Design review of the part shown in the three views and the two pictorial views. Dimensions are in mm from the part's minimum x, y and z. Round coordinates to 2 decimals unless told otherwise and drop trailing zeros. Order: outer loops, then holes, each group sorted by start corner. A loop starts at its lowest first (then second) coordinate and runs counter-clockwise, first axis right, second up.
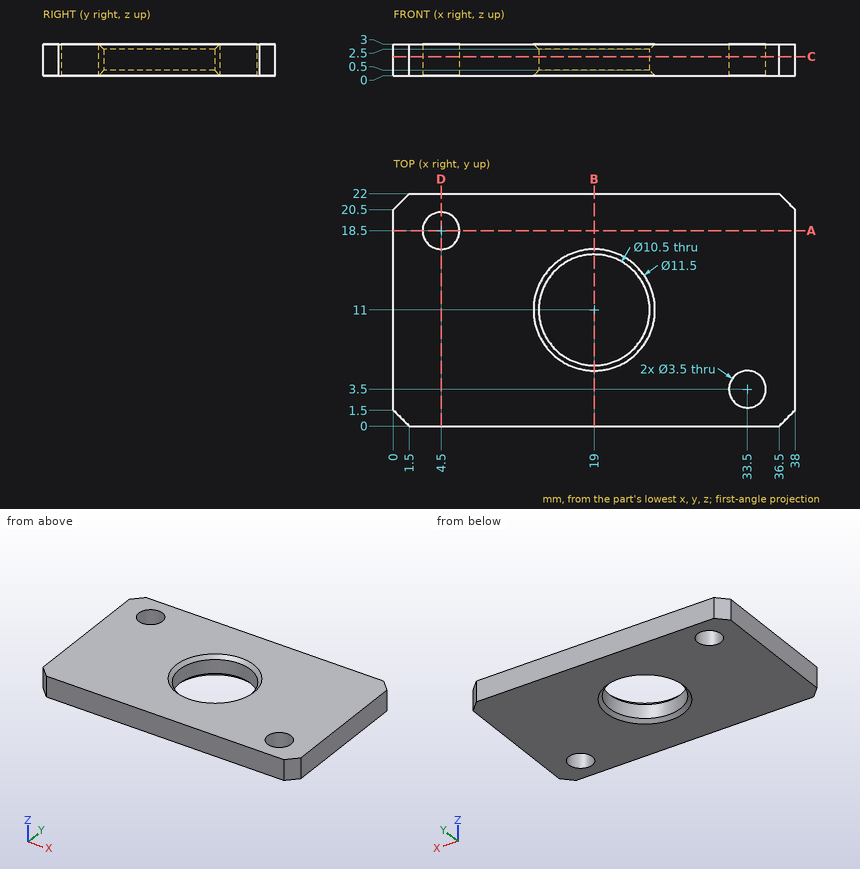
(1) Clearance check with a flat-ended pin moving along its axis: P1, Ø1, axis at x = 6, z = 0.5, coming from the -Y side. State where the tip first meets the part, or that it passes through.
(2) Add section A-A on y = 18.5. Give the boundary of the cut face in (x, z), plus the area to 4 significant figures.
(3) Add section B-B on x = 19. Give the boundary of the cut face in (y, z).
(4) Wall thickness on L1, parallel to Y at x = 33.5, z = 1.75; L2, parallel to Y at x = 19, z = 1.65; L3, parallel to X at y = 13.5, z = 2.5: over which ranges is each line inside the solid? List them lowest first.
(5) Add section C-C on z = 1.8. Give the boundary of the cut face in (x, y).
(6) Add section D-D on x = 4.5. Give the boundary of the cut face in (y, z).
Here are the results:
1. P1: stops at y = 0
2. outline: (0, 0) - (2.75, 0) - (2.75, 3) - (0, 3) - close; (6.25, 0) - (38, 0) - (38, 3) - (6.25, 3) - close
2. area: 103.5 mm2
3. outline: (0, 0) - (5.25, 0) - (5.75, 0.5) - (5.75, 2.5) - (5.25, 3) - (0, 3) - close; (16.25, 0.5) - (16.75, 0) - (22, 0) - (22, 3) - (16.75, 3) - (16.25, 2.5) - close
4. L1: y = 0 to 1.75, 5.25 to 22
4. L2: y = 0 to 5.75, 16.25 to 22
4. L3: x = 0 to 14.38, 23.62 to 38
5. outline: (0, 1.5) - (1.5, 0) - (36.5, 0) - (38, 1.5) - (38, 20.5) - (36.5, 22) - (1.5, 22) - (0, 20.5) - close; hole circle Ø3.5 at (4.5, 18.5); hole circle Ø10.5 at (19, 11); hole circle Ø3.5 at (33.5, 3.5)
6. outline: (0, 0) - (16.75, 0) - (16.75, 3) - (0, 3) - close; (20.25, 0) - (22, 0) - (22, 3) - (20.25, 3) - close
